from build123d import *

# Parameters (mm, degrees)
EXTRUDE_1_DEPTH = 275


with BuildPart() as part:
    # 草图1 → 拉伸-薄壁1 (new, symmetric)
    with BuildSketch(Plane.XY):
        with BuildLine():
            Line((-45, 25), (45, 25))
            ThreePointArc((45, 25), (48.535533906, 23.535533906), (50, 20))
            Line((50, 20), (50, -20))
            ThreePointArc((50, -20), (48.535533906, -23.535533906), (45, -25))
            Line((45, -25), (-45, -25))
            ThreePointArc((-45, -25), (-48.535533906, -23.535533906), (-50, -20))
            Line((-50, -20), (-50, 20))
            ThreePointArc((-50, 20), (-48.535533906, 23.535533906), (-45, 25))
        make_face()
        with BuildLine():
            Line((-45, 21), (45, 21))
            ThreePointArc((45, 21), (45.707106781, 20.707106781), (46, 20))
            Line((46, 20), (46, -20))
            ThreePointArc((46, -20), (45.707106781, -20.707106781), (45, -21))
            Line((45, -21), (-45, -21))
            ThreePointArc((-45, -21), (-45.707106781, -20.707106781), (-46, -20))
            Line((-46, -20), (-46, 20))
            ThreePointArc((-46, 20), (-45.707106781, 20.707106781), (-45, 21))
        make_face(mode=Mode.SUBTRACT)
    extrude(amount=EXTRUDE_1_DEPTH, both=True)


solid = part.part
Geometry check sheet. Reference: the model listing, model coordinates, mm. A direction names the side the tool comes from. Give positions to 0.01 mm unless a question says otherwise; leave off trailing zeros. Write each loop counter-clockwise with the first axis right and the second up, starting at its lowest first coordinate (ties: lowest second). Pieces come first, ordered by that corner, then holes. Notation, with made-up numbers: M 58.5,28 L 65.5,28 A35 cw 65.5,62 Z; hole C 76,88 d5. An arc over 180 degrees is marked long. One line per question, with ' | ' between items.
1. Cross-section at B-B (y = 9). Enter the section's corners in (x, z), plus the area to 3 significant figures.
Ans:
outline: M -50,-275 L -46,-275 L -46,275 L -50,275 Z; M 46,-275 L 50,-275 L 50,275 L 46,275 Z | area: 4,400 mm2
2. Scan lines: line 1 along Y through (x, z) = (-16.5, -236.5); line 2 along X through (y, z) = (0, 227); line 3 along X through (y, z) = (-21.5, -175.5). Record each from-to range of solid material in increasing order. Write a range as from..to.
Ans:
line 1: -25..-21, 21..25 | line 2: -50..-46, 46..50 | line 3: -49.77..49.77
3. Cross-section at A-A (x = 6). Enter the section's corners in (y, z), plus the area to 3 significant figures.
Ans:
outline: M -25,-275 L -21,-275 L -21,275 L -25,275 Z; M 21,-275 L 25,-275 L 25,275 L 21,275 Z | area: 4,400 mm2
4. Set-up check for faces 1 (the face through (46, 0, 4)), 2 (the face through (0, -22, -275)): record each of +Z, -Z, +X, -X, +Y, -Y from which the full face is reachable in a straight line by a thin tool's end or side.
Ans:
face 1: +Z, -Z | face 2: -Z, +X, -X, +Y, -Y
5. Cross-section at C-C (z = -50). Enter the section's corners in (x, y), plus the area to 3 significant figures.
Ans:
outline: M -50,-20 A5 ccw -45,-25 L 45,-25 A5 ccw 50,-20 L 50,20 A5 ccw 45,25 L -45,25 A5 ccw -50,20 Z; hole M -46,-20 A1 ccw -45,-21 L 45,-21 A1 ccw 46,-20 L 46,20 A1 ccw 45,21 L -45,21 A1 ccw -46,20 Z | area: 1,120 mm2
6. Mould release check, pull along X, two halves, no side actions. Record for faces 3 (the face through (50, 0, 4)), 4 (the face through (-46, 0, 4)), 5 (the face through (1, -21, 4)), 6 (the face through (-1, 25, 4)): released by +X, released by -X, zero draft, split by the parting line, or undercut.
Ans:
face 3: released by +X | face 4: undercut | face 5: undercut | face 6: zero draft
